from build123d import *

# Parameters (mm, degrees)
SKETCH_1_R      = 14
SKETCH_1_R_2    = 9
EXTRUDE_1_DEPTH = 16
CHAMFER_1_SIZE  = 0.5


with BuildPart() as part:
    # 草图1 → 拉伸1 (new body)
    with BuildSketch(Plane(origin=(0, 0, 0), x_dir=(1, 0, 0), z_dir=(0, 1, 0))):
        with Locations(Location((0, 0, 0), (0, 0, 270))):
            Circle(SKETCH_1_R)
        with Locations(Location((0, 0, 0), (0, 0, 270))):
            Circle(SKETCH_1_R_2, mode=Mode.SUBTRACT)
    extrude(amount=EXTRUDE_1_DEPTH)

    # 倒角1
    chamfer_1_edges = [part.edges().sort_by_distance(p)[0] for p in [
        (0, 0, -14),
        (0, 16, -14),
        (0, 0, -9),
        (0, 16, -9),
    ]]
    chamfer(chamfer_1_edges, length=CHAMFER_1_SIZE)


solid = part.part
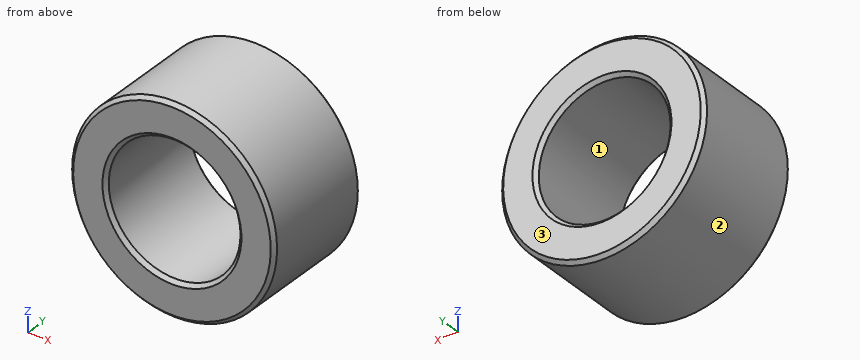
CAD build for the part. Positions are in the model's coordinates, mm. Face numbers are marked on the shaded views. Coordinates: 2 decimals unless noted, no trailing zeros. Order: outer loops, then holes, each group sorted by start corner. A loop starts at its lowest first (then second) coordinate and runs counter-clockwise, first axis right, second up.
Item 1: Drill centre lines: L1, parallel to X at y = 3.75, z = 0; L2, parallel to Z at x = 5.5, y = 11.5; L3, parallel to Z at x = -1.5, y = 10. Where is each one in solid material? Low to high.
Check sheet entries:
L1: x = -14 to -9, 9 to 14
L2: z = -12.87 to -7.12, 7.12 to 12.87
L3: z = -13.92 to -8.87, 8.87 to 13.92
Item 2: Band-saw the part on A-A on x = 0. List the corners of the cut face in (y, z).
Check sheet entries:
outline: (0, -13.5) - (0.5, -14) - (15.5, -14) - (16, -13.5) - (16, -9.5) - (15.5, -9) - (0.5, -9) - (0, -9.5) - close; (0, 9.5) - (0.5, 9) - (15.5, 9) - (16, 9.5) - (16, 13.5) - (15.5, 14) - (0.5, 14) - (0, 13.5) - close
Item 3: Pin check, flat tips, straight feed: pin 1 Ø2 at (x, y) = (-2, 6.5) entering from -Z; pin 2 Ø6 at (x, y) = (11, 4.5) entering from +Z; pin 3 Ø8 at (y, z) = (13, -9.5) entering from -X; pin 4 Ø6 at (x, z) = (0.5, -4.5) entering from +Y. Stop position of each tip, or through.
Check sheet entries:
pin 1: stops at z = -13.96
pin 2: stops at z = 11.49
pin 3: stops at x = -12.87
pin 4: passes through
Item 4: Band-saw the part on B-B on z = 0. List the corners of the cut face in (x, y), plus the area to 3 significant figures.
Check sheet entries:
outline: (-14, 0.5) - (-13.5, 0) - (-9.5, 0) - (-9, 0.5) - (-9, 15.5) - (-9.5, 16) - (-13.5, 16) - (-14, 15.5) - close; (9, 0.5) - (9.5, 0) - (13.5, 0) - (14, 0.5) - (14, 15.5) - (13.5, 16) - (9.5, 16) - (9, 15.5) - close
area: 159 mm2
Item 5: Band-saw the part on C-C on y = 8.5. List the corners of the cut face in (x, z).
Check sheet entries:
outline: circle Ø28 at (0, 0); hole circle Ø18 at (0, 0)
Item 6: Two-plate mould, pull along X, no slides. Class the marked faces 1, 2 and 3: +X half, -X half, draft (parallel to the pull), parting line (faces both ways), or undercut.
Check sheet entries:
face 1: undercut
face 2: parting line
face 3: draft
